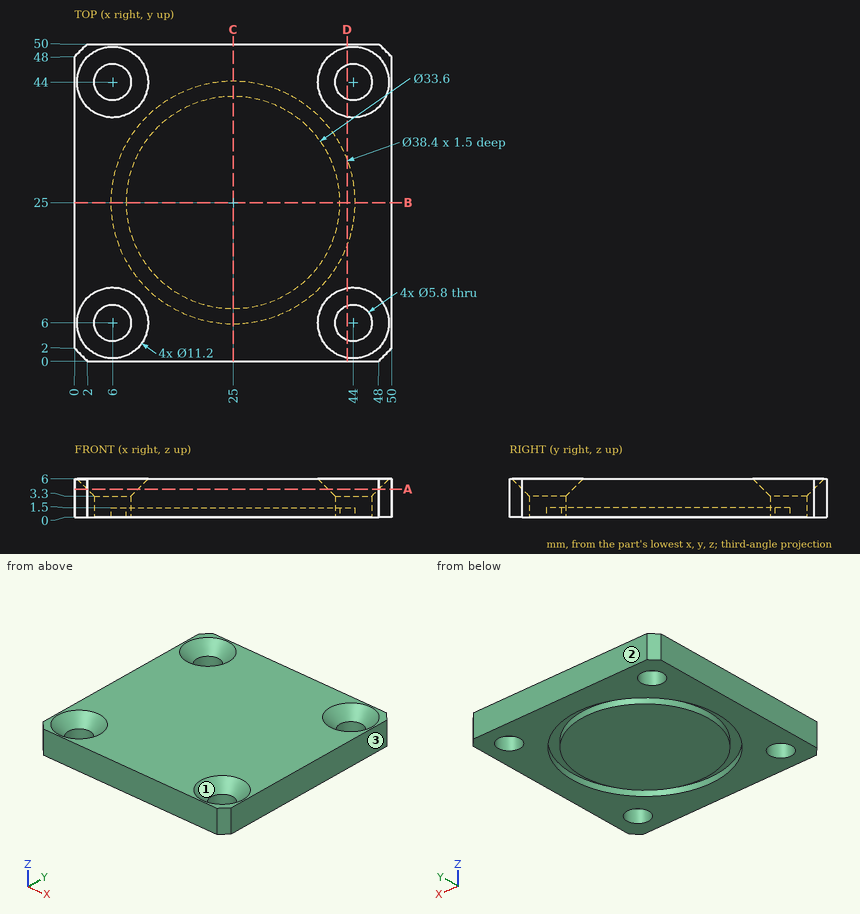
Check sheet for the drawn part. Datum: minimum x, y, z corner. Units: mm. Coordinates: 2 decimals unless noted, no trailing zeros. Order: outer loops, then holes, each group sorted by start corner. A loop starts at its lowest first (then second) coordinate and runs counter-clockwise, first axis right, second up. Notation, with made-up numbers: M -17,-34 L -10,-34 A11 cw -10,-17 Z; hole C 60.5,-12 d4. An arc over 180 degrees is marked long. One line per item, written item: value. Start each with the question number.
Item 1: Gauge pin test, flat end, axial feed: pin 1 (4.5 mm diameter, centred on x = 44, y = 6, fed in from +Z). Record the tip position at first contact, or that the pin passes through.
Item 2: Sectioned sample at D-D (x = 43). Count the separate pieces of the cut face and the enclosed holes in it, then the cut area to 3 significant figures.
Item 3: Mould release check, pull along X, two halves, no side actions. Record for the marked faces 1, 2 and 3: released by +X, released by -X, zero draft, split by the parting line, or undercut.
Item 4: Scan lines: probe 1 along X at (y, z) = (6, 2.2); probe 2 along Y at (x, z) = (25, 0.75); probe 3 along Y at (x, z) = (45, 5.25). Record each from-to range of solid material in increasing order.
Item 5: Sectioned sample at A-A (z = 4.4). Enter the section's corners in (x, y), then the cut area to 3 significant figures.
Item 6: Sectioned sample at B-B (y = 25). Enter the section's corners in (x, z), then the cut area to 3 significant figures.
Conclusion:
1. pin 1: passes through
2. separate pieces: 3
2. enclosed holes: 0
2. area: 199 mm^2
3. face 1: undercut
3. face 2: zero draft
3. face 3: released by +X
4. probe 1: x = 0 to 3.1, 8.9 to 41.1, 46.9 to 50
4. probe 2: y = 0 to 5.8, 8.2 to 41.8, 44.2 to 50
4. probe 3: y = 0 to 1.25, 10.75 to 39.25, 48.75 to 50
5. outline: M 0,2 L 2,0 L 48,0 L 50,2 L 50,48 L 48,50 L 2,50 L 0,48 Z; hole C 6,6 d8; hole C 6,44 d8; hole C 44,6 d8; hole C 44,44 d8
5. area: 2,290 mm^2
6. outline: M 0,0 L 5.8,0 L 5.8,1.5 L 8.2,1.5 L 8.2,0 L 41.8,0 L 41.8,1.5 L 44.2,1.5 L 44.2,0 L 50,0 L 50,6 L 0,6 Z
6. area: 293 mm^2
